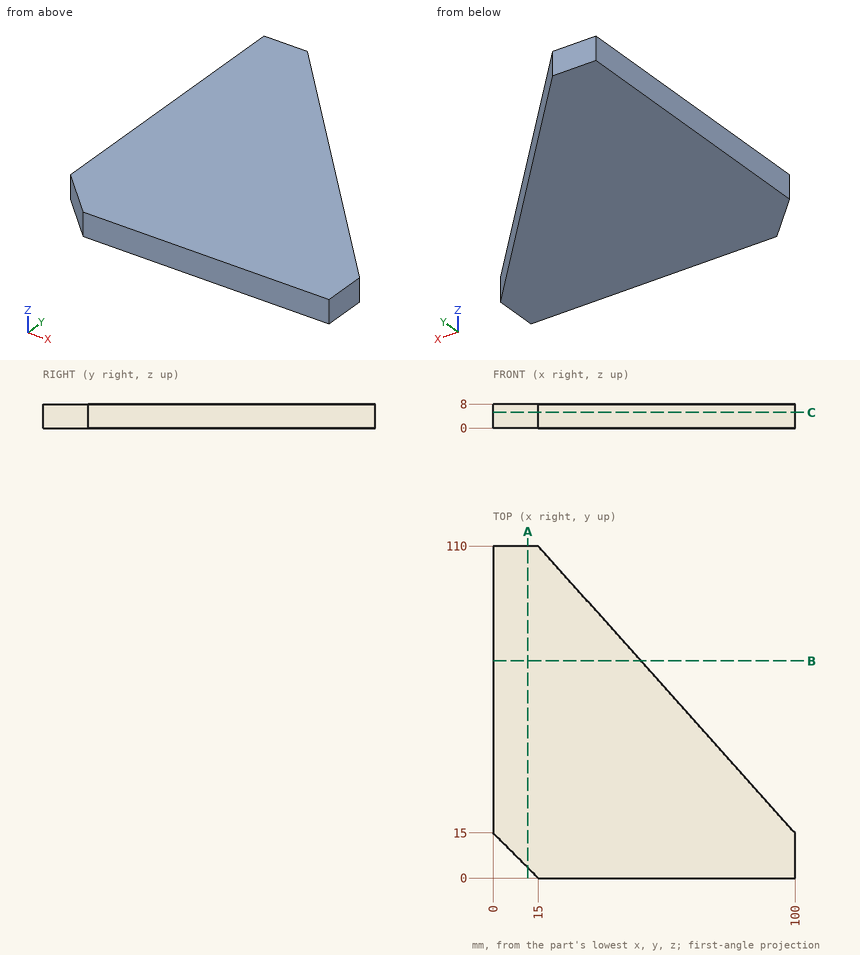
The drawing under review shows one solid part. Ordinate dimensions are in mm from its lowest x, y, z. Coordinates: 2 decimals unless noted, no trailing zeros. Order: outer loops, then holes, each group sorted by start corner. A loop starts at its lowest first (then second) coordinate and runs counter-clockwise, first axis right, second up. Notation, with made-up numbers: (18, 15) -> (70, 15) arc R18 ccw to (70, 36) -> close; hole circle Ø10 at (55, 14). An arc over 180 degrees is marked (long way). Answer in a Markdown table with one row per item.
(1) Consider section C-C (z = 5.25). Write out the cut boundary in (x, y).
Answers:
| item | result |
|---|---|
| outline | (0, 15) -> (15, 0) -> (100, 0) -> (100, 15) -> (15, 110) -> (0, 110) -> close |
(2) Insertion check: pin 1 (2 mm diameter, centred on y = 43, z = 1, fed in from +X); pin 2 (4 mm diameter, centred on y = 24, z = 2, fed in from +X); pin 3 (2 mm diameter, centred on y = 17.5, z = 6, fed in from +X). Each pin has a flat end and moves straight along its axis. Give the tip position at first contact, or say it passes through.
Answers:
| item | result |
|---|---|
| pin 1 | x = 75.84 |
| pin 2 | x = 93.74 |
| pin 3 | x = 98.66 |
(3) Consider section B-B (y = 72). Write out the cut boundary in (x, z).
Answers:
| item | result |
|---|---|
| outline | (0, 0) -> (49, 0) -> (49, 8) -> (0, 8) -> close |
(4) Wall thickness on line 1 along Y through (x, z) = (82.5, 3.5); line 2 along Y through (x, z) = (37, 1.75); line 3 along X through (y, z) = (89.5, 3.75): over which ranges is each line inside the solid? List them lowest first.
Answers:
| item | result |
|---|---|
| line 1 | 0 to 34.56 |
| line 2 | 0 to 85.41 |
| line 3 | 0 to 33.34 |
(5) Consider section A-A (x = 11.5). Write out the cut boundary in (y, z).
Answers:
| item | result |
|---|---|
| outline | (3.5, 0) -> (110, 0) -> (110, 8) -> (3.5, 8) -> close |
